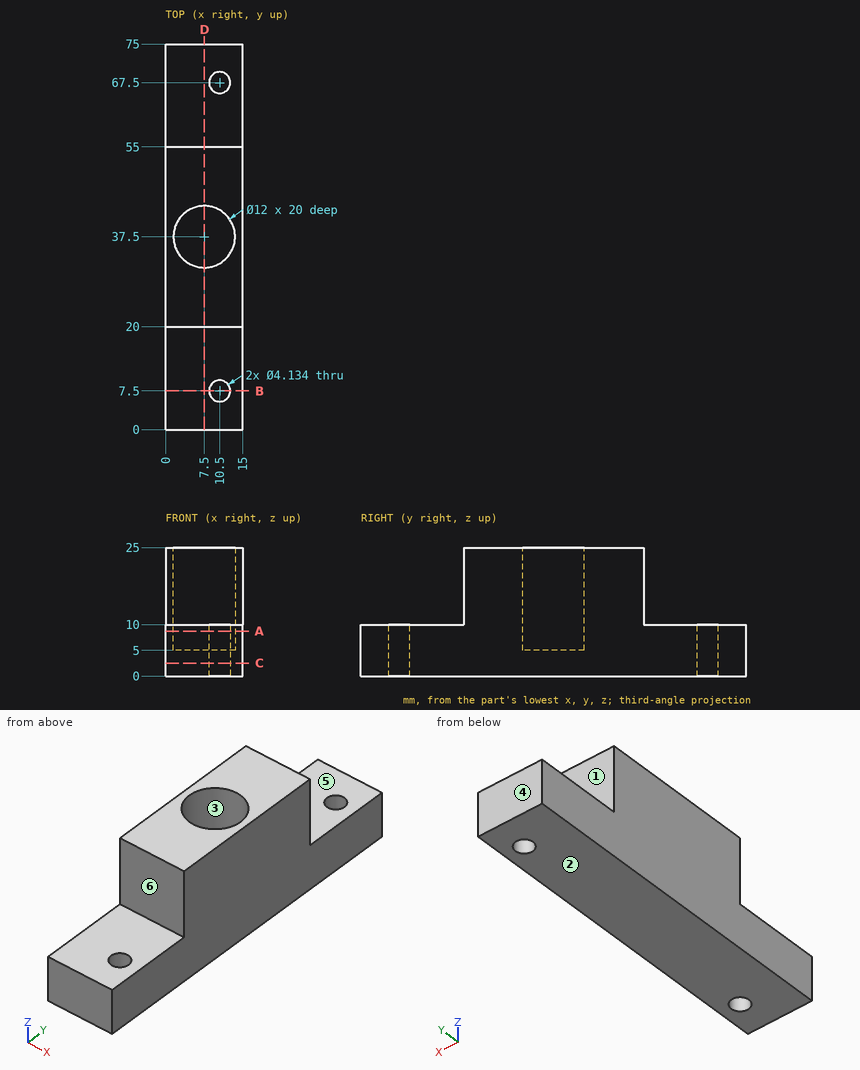
The figure shows three views and two pictorial views of one solid part (mm, origin at its lowest corner). Answer the questions. A direction names the side the tool comes from. Round coordinates to 2 decimals unless told otherwise and drop trailing zeros. Write each loop counter-clockwise with the first axis right and the second up, starting at its lowest first coordinate (ties: lowest second). Pieces come first, ordered by that corner, then holes. Notation, with made-up numbers: M 66,30 L 70,30 A21 ccw 70,47 Z; hole C -15.5,46 d10. An arc over 180 degrees is marked long. Use a Markdown table: item, result.
1) A tool of negligible diameter and unlimited length cuts with its end or side. For the marked faces 4, 5 and 6, from which of +Z, -Z, +X, -X, +Y, -Y can it reach the whole face along a straight path? Write none if from no direction.
Answers follow:
| item | result |
|---|---|
| face 4 | +Z, -Z, +X, -X, +Y |
| face 5 | +Z, +X, -X, +Y |
| face 6 | +Z, +X, -X, -Y |
2) The part is cut by section B-B (y = 7.5). Write down the section's boundary in (x, z), plus the area to 3 significant figures.
Answers follow:
| item | result |
|---|---|
| outline | M 0,0 L 8.43,0 L 8.43,10 L 0,10 Z; M 12.57,0 L 15,0 L 15,10 L 12.57,10 Z |
| area | 109 mm2 |
3) For a pull along Y with two mould halves and no side action, classify the marked faces 1, 2 and 3 as pulls with the +Y half, pulls with the -Y half, needs draft (parallel to the pull), parting line crosses it, or undercut.
Answers follow:
| item | result |
|---|---|
| face 1 | pulls with the +Y half |
| face 2 | needs draft |
| face 3 | undercut |
4) The part is cut by section C-C (z = 2.5). Write down the section's boundary in (x, y).
Answers follow:
| item | result |
|---|---|
| outline | M 0,0 L 15,0 L 15,75 L 0,75 Z; hole C 10.5,7.5 d4.13; hole C 10.5,67.5 d4.13 |
5) Straight lines are drawn through the part: line 1 along Y through (x, z) = (10.5, 3); line 2 along Y through (x, z) = (7.75, 20.5); line 3 along Y through (x, z) = (9.5, 1.75). For each, find the intervals that lie inside material, in ascending order. Write a range as [from, to].
Answers follow:
| item | result |
|---|---|
| line 1 | y = [0, 5.43], [9.57, 65.43], [69.57, 75] |
| line 2 | y = [20, 31.51], [43.49, 55] |
| line 3 | y = [0, 5.69], [9.31, 65.69], [69.31, 75] |
6) The part is cut by section D-D (x = 7.5). Write down the section's boundary in (y, z).
Answers follow:
| item | result |
|---|---|
| outline | M 0,0 L 75,0 L 75,10 L 55,10 L 55,25 L 43.5,25 L 43.5,5 L 31.5,5 L 31.5,25 L 20,25 L 20,10 L 0,10 Z |
7) Flat-ended cylindrical pins translate along their axes: pin 1 (4.5 mm diameter, centred on x = 7.5, z = 14.5, fed in from -Y); pin 2 (8 mm diameter, centred on x = 9.5, z = 15, fed in from +Y); pin 3 (5 mm diameter, centred on x = 10.5, y = 7.5, fed in from +Z). Find the tip coordinate at first contact, or state that the pin passes through.
Answers follow:
| item | result |
|---|---|
| pin 1 | stops at y = 20 |
| pin 2 | stops at y = 55 |
| pin 3 | stops at z = 10 |
8) The part is cut by section A-A (z = 8.75). Write down the section's boundary in (x, y), plus the area to 3 significant figures.
Answers follow:
| item | result |
|---|---|
| outline | M 0,0 L 15,0 L 15,75 L 0,75 Z; hole C 7.5,37.5 d12; hole C 10.5,7.5 d4.13; hole C 10.5,67.5 d4.13 |
| area | 985 mm2 |
